Part model, mm, in its own coordinate system. A direction names the side the tool comes from. Give positions to 0.01 mm unless a question says otherwise; leave off trailing zeros. Order: outer loops, then holes, each group sorted by start corner. A loop starts at its lowest first (then second) coordinate and runs counter-clockwise, first axis right, second up.
from build123d import *

# Parameters (mm, degrees)
BOSS_EXTRUDE1_DEPTH                                  = 25
CHAMFER1_SIZE                                        = 0.5
HOLE_SIZE_PER_SOCKET_HEAD_CAP_SCREW_TYPE_D           = 3.4
HOLE_SIZE_PER_SOCKET_HEAD_CAP_SCREW_TYPE_CBORE_D     = 6
HOLE_SIZE_PER_SOCKET_HEAD_CAP_SCREW_TYPE_CBORE_DEPTH = 3.4
M3_TAPPED_HOLE1_D                                    = 2.5
M3_TAPPED_HOLE1_DEPTH                                = 7.5
M3_TAPPED_HOLE1_TIP                                  = 0.751075774


with BuildPart() as part:
    # Sketch1 → Boss-Extrude1 (new, symmetric)
    with BuildSketch(Plane(origin=(0, 0, 0), x_dir=(1, 0, 0), z_dir=(0, 1, 0))):
        Polygon((0, 0), (40, 0), (40, 5.5), (27, 5.5), (27, 6), (13, 6), (13, 5.5), (0, 5.5), align=None)
    extrude(amount=BOSS_EXTRUDE1_DEPTH, both=True)

    # Chamfer1
    chamfer1_edges = [part.edges().sort_by_distance(p)[0] for p in [
        (0, 0, -5.5),
        (40, 0, -5.5),
        (40, 0, 0),
        (0, 0, 0),
    ]]
    chamfer(chamfer1_edges, length=CHAMFER1_SIZE)

    # Hole Size per Socket Head Cap Screw Type1 (through all)
    with Locations(Plane.XY):
        with Locations((20, -7.5), (20, -17.5)):
            CounterBoreHole(HOLE_SIZE_PER_SOCKET_HEAD_CAP_SCREW_TYPE_D / 2, HOLE_SIZE_PER_SOCKET_HEAD_CAP_SCREW_TYPE_CBORE_D / 2, HOLE_SIZE_PER_SOCKET_HEAD_CAP_SCREW_TYPE_CBORE_DEPTH)

    # M3 Tapped Hole1
    with Locations(Plane.XY):
        with Locations((20, 13), (29, 13), (20, 4), (29, 4)):
            Hole(M3_TAPPED_HOLE1_D / 2, depth=M3_TAPPED_HOLE1_DEPTH)
            with Locations((0, 0, -(M3_TAPPED_HOLE1_DEPTH + M3_TAPPED_HOLE1_TIP / 2))):  # 118° drill point
                Cone(0, M3_TAPPED_HOLE1_D / 2, M3_TAPPED_HOLE1_TIP, mode=Mode.SUBTRACT)


solid = part.part
Item 1: Band-saw the part on C-C on y = 4. List the corners of the cut face in (x, z).
Item 2: Drop flat-ended pins along their axis: P1, Ø1.8, axis at x = 19.5, y = -18.5, coming from the +Z side; P2, Ø6, axis at x = 8, y = -4, coming from the -Z side; P3, Ø1.5, axis at x = 29, y = 13, coming from the -Z side. Give the stop position or say it passes through.
Item 3: Which spindle directions (+Z, -Z, +X, -X, +Y, -Y) get a long thin tool onto all of the face, cutting with end or side? Do faces 4 (the face through (33, 0, -5.5)), 5 (the face through (18.43, -8.15, -4.72)), 6 (the face through (17.79, -5.47, -1.68)). Say none if no direction does.
Item 4: Band-saw the part on B-B on x = 20. List the corners of the cut face in (y, z).
Item 5: Pull direction Y, two halves, no side cores. Call faces 1 (the face through (7, 0, -5.5)), 2 (the face through (19.328, 14.054, -3.042)), 3 (the face through (20, 25, -3)): released by +Y, released by -Y, zero draft, split by the parting line, or undercut.
Item 6: Band-saw the part on A-A on y = -7.5. List the corners of the cut face in (x, z).
Item 7: Band-saw the part on D-D on z = -1.15. List the corners of the cut face in (x, y).
Item 8: Drill centre lines: probe 1 along Y at (x, z) = (20, -1.15); probe 2 along Y at (x, z) = (29, -1.65); probe 3 along Y at (x, z) = (20, -4.5). Where is each one in solid material? Low to high.
Working result:
1. outline: (0, -5) - (0.5, -5.5) - (13, -5.5) - (13, -6) - (18.75, -6) - (18.75, 0) - (0.5, 0) - (0, -0.5) - close; (21.25, -6) - (27, -6) - (27, -5.5) - (27.75, -5.5) - (27.75, 0) - (21.25, 0) - close; (30.25, -5.5) - (39.5, -5.5) - (40, -5) - (40, -0.5) - (39.5, 0) - (30.25, 0) - close
2. P1: stops at z = -3.4
2. P2: stops at z = -5.5
2. P3: passes through
3. face 4: -Z, +X, +Y, -Y
3. face 5: +Z, -Z
3. face 6: +Z
4. outline: (-25, -6) - (-19.2, -6) - (-19.2, -3.4) - (-20.5, -3.4) - (-20.5, 0) - (-25, 0) - close; (-15.8, -6) - (-9.2, -6) - (-9.2, -3.4) - (-10.5, -3.4) - (-10.5, 0) - (-14.5, 0) - (-14.5, -3.4) - (-15.8, -3.4) - close; (-5.8, -6) - (2.75, -6) - (2.75, 0) - (-4.5, 0) - (-4.5, -3.4) - (-5.8, -3.4) - close; (5.25, -6) - (11.75, -6) - (11.75, 0) - (5.25, 0) - close; (14.25, -6) - (25, -6) - (25, 0) - (14.25, 0) - close
5. face 1: zero draft
5. face 2: undercut
5. face 3: released by +Y
6. outline: (0, -5) - (0.5, -5.5) - (13, -5.5) - (13, -6) - (18.3, -6) - (18.3, -3.4) - (17, -3.4) - (17, 0) - (0.5, 0) - (0, -0.5) - close; (21.7, -6) - (27, -6) - (27, -5.5) - (39.5, -5.5) - (40, -5) - (40, -0.5) - (39.5, 0) - (23, 0) - (23, -3.4) - (21.7, -3.4) - close
7. outline: (0, -25) - (40, -25) - (40, 25) - (0, 25) - close; hole circle Ø6 at (20, -17.5); hole circle Ø6 at (20, -7.5); hole circle Ø2.5 at (20, 4); hole circle Ø2.5 at (20, 13); hole circle Ø2.5 at (29, 4); hole circle Ø2.5 at (29, 13)
8. probe 1: y = -25 to -20.5, -14.5 to -10.5, -4.5 to 2.75, 5.25 to 11.75, 14.25 to 25
8. probe 2: y = -25 to 2.75, 5.25 to 11.75, 14.25 to 25
8. probe 3: y = -25 to -19.2, -15.8 to -9.2, -5.8 to 2.75, 5.25 to 11.75, 14.25 to 25
